```python
from build123d import *

# Parameters (mm, degrees)
BOSS_EXTRUDE_1_DEPTH = 800


with BuildPart() as part:
    # Sketch 1 → Boss-Extrude 1 (new, symmetric)
    with BuildSketch(Plane.XY):
        with BuildLine():
            Line((60, 0), (-60, 0))
            Line((-60, 0), (-60, -53))
            ThreePointArc((-60, -53), (-56.980458786, -51.836520772), (-55.522328009, -48.947720382))
            Line((-55.522328009, -48.947720382), (-51.988381432, -13.604559236))
            ThreePointArc((-51.988381432, -13.604559236), (-49.072119877, -7.826958457), (-43.03303745, -5.5))
            Line((-43.03303745, -5.5), (43.03303745, -5.5))
            ThreePointArc((43.03303745, -5.5), (49.072119877, -7.826958457), (51.988381432, -13.604559236))
            Line((51.988381432, -13.604559236), (55.522328009, -48.947720382))
            ThreePointArc((55.522328009, -48.947720382), (56.980458786, -51.836520772), (60, -53))
            Line((60, -53), (60, 0))
        make_face()
    extrude(amount=BOSS_EXTRUDE_1_DEPTH, both=True)


solid = part.part
```
Build history of the part. All positions in model axes, mm. A direction names the side the tool comes from. Round coordinates to 2 decimals unless told otherwise and drop trailing zeros. Loops run counter-clockwise (first coordinate to the right, second up) from the corner with the lowest first, then second, coordinate; pieces in that order, holes last.
Item 1: Which spindle directions (+Z, -Z, +X, -X, +Y, -Y) get a long thin tool onto all of the face, cutting with end or side? Do faces 1 (the face through (-60, -26, 11)), 2 (the face through (-1, -5.5, 11)). Say none if no direction does.
Item 2: Pin check, flat tip, straight feed: P1, Ø10, axis at x = 1.5, z = 152, coming from the +Y side. Stop position of the tip, or through.
Item 3: Saw through at A-A (z = -139). List the corners of the cut face in (x, y), then the cut area to 3 significant figures.
Item 4: Drill centre lines: line 1 along X through (y, z) = (-23, 256); line 2 along Y through (x, z) = (0, -260); line 3 along X through (y, z) = (-34, 440.5). Where is each one in solid material? Low to high.
Item 5: Saw through at B-B (y = -36.5). List the corners of the cut face in (x, z), then the cut area to 3 significant figures.
Item 6: Two-plate mould, pull along X, no slides. Class faces 3 (the face through (0, -5, 800)), 4 (the face through (53.73, -31.03, 11.2)), 5 (the face through (60, -27, 11)): released by +X, released by -X, zero draft, split by the parting line, or undercut.
Item 7: Saw through at C-C (x = 27.5). List the corners of the cut face in (y, z), then the cut area to 3 significant figures.
Worked answers:
1. face 1: +Z, -Z, -X, +Y, -Y
1. face 2: +Z, -Z, -Y
2. P1: stops at y = 0
3. outline: (-60, -53) arc R4.5 ccw to (-55.52, -48.95) - (-51.99, -13.6) arc R9 cw to (-43.03, -5.5) - (43.03, -5.5) arc R9 cw to (51.99, -13.6) - (55.52, -48.95) arc R4.5 ccw to (60, -53) - (60, 0) - (-60, 0) - close
3. area: 1,290 mm2
4. line 1: x = -60 to -52.93, 52.93 to 60
4. line 2: y = -5.5 to 0
4. line 3: x = -60 to -54.03, 54.03 to 60
5. outline: (-60, -800) - (-54.28, -800) - (-54.28, 800) - (-60, 800) - close; (54.28, -800) - (60, -800) - (60, 800) - (54.28, 800) - close
5. area: 18,300 mm2
6. face 3: zero draft
6. face 4: undercut
6. face 5: released by +X
7. outline: (-5.5, -800) - (0, -800) - (0, 800) - (-5.5, 800) - close
7. area: 8,800 mm2
